Drawing for the job (mm, zero at the part's lowest x, y, z). Give positions to 0.01 mm unless a question says otherwise; leave off trailing zeros. Loops run counter-clockwise (first coordinate to the right, second up) from the corner with the lowest first, then second, coordinate; pieces in that order, holes last.
1) Band-saw the part on A-A on y = 27.5. List the corners of the cut face in (x, z).
2) Flat gauge pins, fed straight in: P1, Ø2, axis at y = 33.5, z = 5.5, coming from the -X side; P2, Ø8, axis at x = 19.5, z = 11, coming from the +Y side; P3, Ø3, axis at y = 45.5, z = 7, coming from the +X side. Where does each tip first touch, or does it go through?
3) Two-plate mould, pull along X, no slides. Class the marked faces 1, 2 and 3: +X half, -X half, draft (parallel to the pull), parting line (faces both ways), or undercut.
4) Band-saw the part on C-C on z = 10.75. List the corners of the cut face in (x, y).
5) Wall check: line 1 (Y direction, x = 27.5, z = 11.5); line 2 (Y direction, x = 27.5, z = 7); line 3 (Z direction, x = 4, y = 33). Give the ranges that are in metal, low to high.
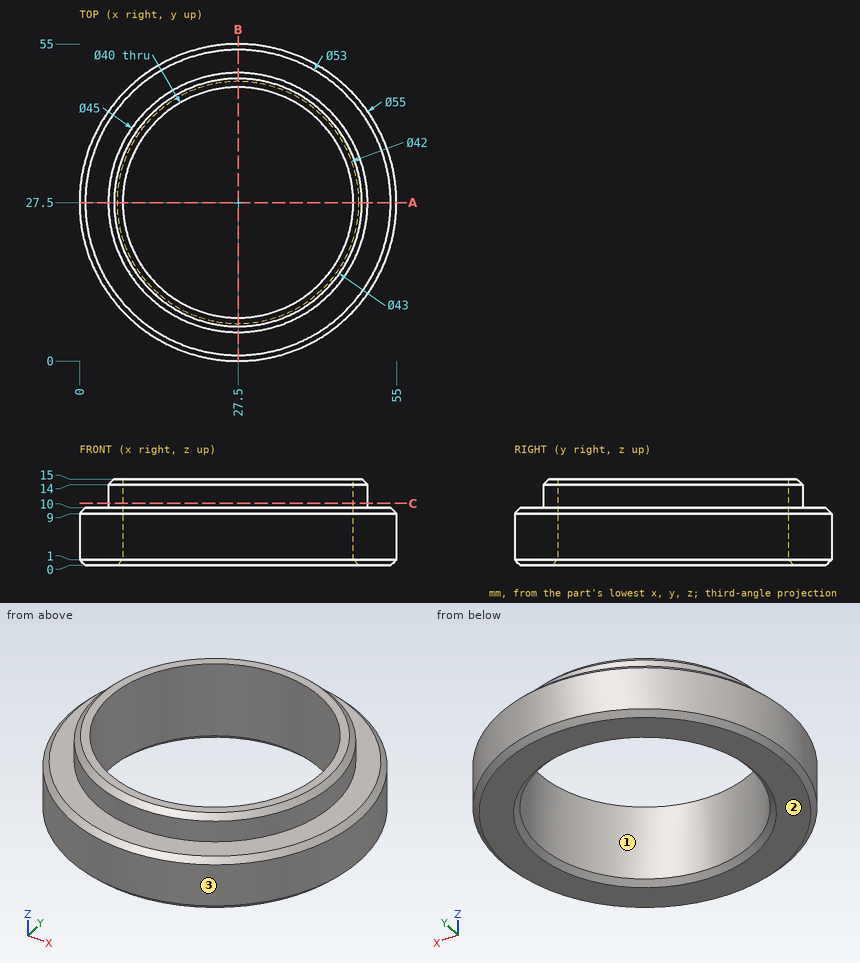
Findings below:
1. outline: (0, 1) - (1, 0) - (6.5, 0) - (7.5, 1) - (7.5, 15) - (6, 15) - (5, 14) - (5, 10) - (1, 10) - (0, 9) - close; (47.5, 1) - (48.5, 0) - (54, 0) - (55, 1) - (55, 9) - (54, 10) - (50, 10) - (50, 14) - (49, 15) - (47.5, 15) - close
2. P1: stops at x = 0.46
2. P2: stops at y = 54.62
2. P3: stops at x = 49.5
3. face 1: undercut
3. face 2: draft
3. face 3: parting line
4. outline: circle Ø45 at (27.5, 27.5); hole circle Ø40 at (27.5, 27.5)
5. line 1: y = 5 to 7.5, 47.5 to 50
5. line 2: y = 0 to 7.5, 47.5 to 55
5. line 3: z = 0 to 10
